```python
from build123d import *

# Parameters (mm, degrees)
SKETCH2_R           = 95
SKETCH2_R_2         = 27.5
BOSS_EXTRUDE1_DEPTH = 10
SKETCH3_R           = 10
CUT_EXTRUDE1_DEPTH  = 135.721935853
CIRPATTERN1_COUNT   = 8


with BuildPart() as part:
    # Sketch2 → Boss-Extrude1 (new body)
    with BuildSketch(Plane.XY):
        Circle(SKETCH2_R)
        Circle(SKETCH2_R_2, mode=Mode.SUBTRACT)
    extrude(amount=BOSS_EXTRUDE1_DEPTH)

    # Sketch3 → Cut-Extrude1 (cut, symmetric)
    with BuildSketch(Plane.XY.offset(10)):
        with Locations((50, 0)):
            Circle(SKETCH3_R)
    cut_extrude1 = extrude(amount=CUT_EXTRUDE1_DEPTH, both=True, mode=Mode.SUBTRACT)

    # CirPattern1: Cut-Extrude1 ×8 about axis
    cirpattern1_axis = Axis((0, 0, 0), (0, 0, 1))
    for i in range(1, CIRPATTERN1_COUNT):
        add(cut_extrude1.rotate(cirpattern1_axis, i * 360 / CIRPATTERN1_COUNT), mode=Mode.SUBTRACT)


solid = part.part
```
Read the model definition and answer for the solid it produces. Units are mm, in the model's axes. Round coordinates to 2 decimals unless told otherwise and drop trailing zeros. Write each loop counter-clockwise with the first axis right and the second up, starting at its lowest first coordinate (ties: lowest second). Pieces come first, ordered by that corner, then holes. Notation, with made-up numbers: M 7.25,83.5 L 20.25,83.5 A35 cw 20.25,119.5 Z; hole C 9,-17 d8. An arc over 180 degrees is marked long. One line per item, written item: value.
Q1. Find section B-B on x = 50. Write down the section's boundary in (y, z).
Data:
outline: M -80.78,0 L -10,0 L -10,10 L -80.78,10 Z; M 10,0 L 80.78,0 L 80.78,10 L 10,10 Z
Q2. Find section D-D on z = 3.5. Count the separate pieces of the cut face and the enclosed holes in it, plus the area to 3 significant figures.
Data:
separate pieces: 1
enclosed holes: 9
area: 23,500 mm2
Q3. Find section A-A on y = 0. Write down the section's boundary in (x, z).
Data:
outline: M -95,0 L -60,0 L -60,10 L -95,10 Z; M -40,0 L -27.5,0 L -27.5,10 L -40,10 Z; M 27.5,0 L 40,0 L 40,10 L 27.5,10 Z; M 60,0 L 95,0 L 95,10 L 60,10 Z
Q4. Flat-ended cylindrical pins translate along their axes: pin 1 Ø18 at (x, y) = (-35.36, -35.36) entering from -Z; pin 2 Ø5 at (x, z) = (-8.5, 5) entering from +Y; pin 3 Ø1 at (y, z) = (-15.5, 7.5) entering from +X; pin 4 Ø4 at (y, z) = (37.5, 4.5) entering from +X. Find the tip coordinate at first contact, or state that the pin passes through.
Data:
pin 1: through
pin 2: y = 94.81
pin 3: x = 93.81
pin 4: x = 88.12
Q5. Straight lines are drawn through the part: line 1 (X direction, y = -2, z = 4.25); line 2 (Y direction, x = 3, z = 9); line 3 (Y direction, x = -4, z = 6). For each, find the intervals that lie inside material, in ascending order. Write a range as [from, to].
Data:
line 1: [-94.98, -59.8], [-40.2, -27.43], [27.43, 40.2], [59.8, 94.98]
line 2: [-94.95, -59.54], [-40.46, -27.34], [27.34, 40.46], [59.54, 94.95]
line 3: [-94.92, -59.17], [-40.83, -27.21], [27.21, 40.83], [59.17, 94.92]
Q6. For a pull along Y with two mould halves and no side action, classify faces 1 (the flat face through (20, -20, 0)), 2 (the cylindrical face through (40, 0, 5)), 3 (the cylindrical face through (-20.59, -92.74, 4.93)), 4 (the cylindrical face through (0, 40, 5)) as +Y half, -Y half, draft (parallel to the pull), parting line (faces both ways), or undercut.
Data:
face 1: draft
face 2: undercut
face 3: parting line
face 4: undercut
